```python
from build123d import *

# Parameters (mm, degrees)
BACK_PLATE_SKETCH_W    = 110
BACK_PLATE_SKETCH_H    = 66
BACK_PLATE_DEPTH       = 10
TOP_BOSS_44_DEPTH      = 20
TOP_BOSS_44_DEPTH_BACK = 20
TOP_BOSS_SKETCH_R      = 22
TOP_BOSS_SKETCH_R_2    = 11
PLATE_CUT_SKETCH_R     = 7.5
PLATE_CUT_DEPTH        = 20
BASE_BLOCK_DEPTH       = 64
BEARING_SADDLE_DEPTH   = 22
EAR_HOLES_SKETCH_R     = 6
EAR_HOLES_12_DEPTH     = 22
RIB_DEPTH              = 10
SIDE_PLATE_DEPTH       = 5
PAD_1_SKETCH_W         = 9.88210357
PAD_1_SKETCH_H         = 10
PAD_1_DEPTH            = 2
PAD_2_SKETCH_W         = 64
PAD_2_SKETCH_H         = 10
PAD_2_DEPTH            = 2


with BuildPart() as part:
    # Back Plate Sketch → Back Plate (new, symmetric)
    with BuildSketch(Plane(origin=(0, 0, 0), x_dir=(0, 0, -1), z_dir=(1, 0, 0))):
        Rectangle(BACK_PLATE_SKETCH_W, BACK_PLATE_SKETCH_H)
    extrude(amount=BACK_PLATE_DEPTH, both=True)

    # Plate Cut Sketch → Plate Cut (cut)
    with BuildSketch(Plane(origin=(10, 0, 0), x_dir=(0, 0, -1), z_dir=(1, 0, 0))):
        with Locations((42.5, 11)):
            Circle(PLATE_CUT_SKETCH_R)
        with Locations(Location((-42.5, 11, 0), (0, 0, 180))):
            Circle(PLATE_CUT_SKETCH_R)
    extrude(amount=-PLATE_CUT_DEPTH, mode=Mode.SUBTRACT)

    # Base Block Sketch → Base Block (add)
    with BuildSketch(Plane(origin=(10, 0, 0), x_dir=(0, 0, -1), z_dir=(1, 0, 0))):
        with BuildLine():
            Line((-32, -33), (-18, -33))
            ThreePointArc((-18, -33), (0, -15), (18, -33))
            Line((18, -33), (32, -33))
            ThreePointArc((32, -33), (0, -1), (-32, -33))
        make_face()
    extrude(amount=BASE_BLOCK_DEPTH)

    # Bearing Saddle Sketch → Bearing Saddle (add)
    with BuildSketch(Plane.XZ.offset(33)):
        with BuildLine():
            Line((27, 38), (27, 18))
            Line((27, 18), (57, 18))
            Line((57, 18), (57, 38))
            ThreePointArc((57, 38), (42, 53), (27, 38))
        make_face()
        with BuildLine():
            Line((27, -38), (27, -18))
            Line((27, -18), (57, -18))
            Line((57, -18), (57, -38))
            ThreePointArc((57, -38), (42, -53), (27, -38))
        make_face()
    extrude(amount=-BEARING_SADDLE_DEPTH)

    # Ear Holes Sketch → Ear Holes Ø12 (cut)
    with BuildSketch(Plane(origin=(0, -11, 0), x_dir=(1, 0, 0), z_dir=(0, 1, 0))):
        with Locations(Location((42, 38, 0), (0, 0, 270))):
            Circle(EAR_HOLES_SKETCH_R)
        with Locations(Location((42, -38, 0), (0, 0, 270))):
            Circle(EAR_HOLES_SKETCH_R)
    extrude(amount=-EAR_HOLES_12_DEPTH, mode=Mode.SUBTRACT)



with BuildPart() as body_2:
    # Top Boss Sketch → Top Boss Ø44 (new, two sides: drawn at the far end of the back side and taken through both)
    with BuildSketch(Plane(origin=(0, 0, 0), x_dir=(0, 0, -1), z_dir=(1, 0, 0)).offset(-TOP_BOSS_44_DEPTH_BACK)):
        with Locations((0, 67)):
            Circle(TOP_BOSS_SKETCH_R)
        with Locations((0, 67)):
            Circle(TOP_BOSS_SKETCH_R_2, mode=Mode.SUBTRACT)
    extrude(amount=TOP_BOSS_44_DEPTH + TOP_BOSS_44_DEPTH_BACK)


with BuildPart() as part_1:
    add(part.part)

    add(body_2.part)  # Rib merges body 2
    # Rib Sketch → Rib (add)
    with BuildSketch(Plane(origin=(10, 0, 0), x_dir=(0, 0, -1), z_dir=(1, 0, 0))):
        with BuildLine():
            Line((-22, 67), (-55, 33))
            Line((-55, 33), (55, 33))
            Line((55, 33), (22, 67))
            ThreePointArc((22, 67), (0, 45), (-22, 67))
        make_face()
    extrude(amount=-RIB_DEPTH)

    # Side Plate Sketch → Side Plate (add, symmetric)
    with BuildSketch(Plane.XY):
        Polygon((10, 44), (19.88210357, 44), (74, 0), (10, 0), align=None)
    extrude(amount=SIDE_PLATE_DEPTH, both=True)

    # Pad 1 Sketch → Pad 1 (add)
    with BuildSketch(Plane(origin=(0, 44, 0), x_dir=(1, 0, 0), z_dir=(0, 1, 0))):
        with Locations((14.941051785, 0)):
            Rectangle(PAD_1_SKETCH_W, PAD_1_SKETCH_H)
    extrude(amount=PAD_1_DEPTH)

    # Pad 2 Sketch → Pad 2 (add)
    with BuildSketch(Plane.XZ):
        with Locations((42, 0)):
            Rectangle(PAD_2_SKETCH_W, PAD_2_SKETCH_H)
    extrude(amount=PAD_2_DEPTH)


solid = part_1.part
```
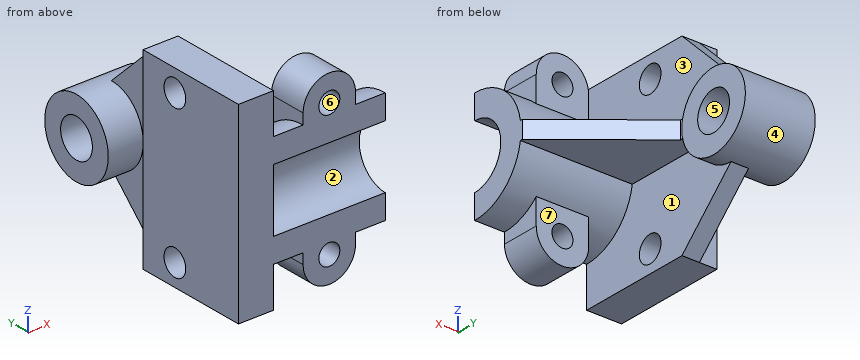
The model under review builds one solid part; all positions refer to its coordinate system, in mm. Face numbers are marked on the shaded views. A direction names the side the tool comes from. Give positions to 0.01 mm unless a question says otherwise; leave off trailing zeros. Loops run counter-clockwise (first coordinate to the right, second up) from the corner with the lowest first, then second, coordinate; pieces in that order, holes last. Notation, with made-up numbers: (81, -7.75) - (117, -7.75) arc R19 ccw to (117, 10.25) - close; hole circle Ø4 at (86, 21). An arc over 180 degrees is marked (long way). Answer as a JSON object with one key per item and string values.
Q1. To check wall thickness, follow line 1 along Y through (x, z) = (-6, 0); line 2 along Z through (x, y) = (3, 12.5); line 3 along Y through (x, z) = (15, -6). State the ranges of each line that lie inside material, in increasing order.
Worked out:
{"line 1": "y = -33 to 33, 45 to 56, 78 to 89", "line 2": "z = -55 to -49.85, -35.15 to 35.15, 49.85 to 55", "line 3": "y = -16.03 to -1.57, 45.83 to 57.78, 76.22 to 88.17"}
Q2. Insertion check: pin 1 (15 mm diameter, centred on x = 46.5, z = -43, fed in from +Y); pin 2 (15 mm diameter, centred on y = 12.5, z = 39, fed in from +X); pin 3 (5 mm diameter, centred on y = 9, z = 5, fed in from -X). Each pin has a flat end and moves straight along its axis. Give the tip position at first contact, or say it passes through.
Worked out:
{"pin 1": "stops at y = -11", "pin 2": "stops at x = 10", "pin 3": "stops at x = -10"}
Q3. Add section D-D on y = 62.5. State the section outline as (x, z) points, plus the area to 3 significant figures.
Worked out:
{"outline": "(-20, -21.53) - (0, -21.53) - (0, -26.37) - (10, -26.37) - (10, -21.53) - (20, -21.53) - (20, -10.04) - (-20, -10.04) - close; (-20, 10.04) - (20, 10.04) - (20, 21.53) - (10, 21.53) - (10, 26.37) - (0, 26.37) - (0, 21.53) - (-20, 21.53) - close", "area": "1,020 mm^2"}
Q4. For the marked faces 1, 2 and 3, list the 3-axis set-ups (+Z, -Z, +X, -X, +Y, -Y) from which the entire face can be reached by the end or side of a thin tool; tool diameter is ignored.
Worked out:
{"face 1": "-Z", "face 2": "+X, -Y", "face 3": "+Z"}
Q5. Mouldability with a two-part tool opening along Y and no side actions: class the marked faces 4, 5, 6 and 7 as +Y half, -Y half, draft (parallel to the pull), parting line (faces both ways), or undercut.
Worked out:
{"face 4": "undercut", "face 5": "undercut", "face 6": "draft", "face 7": "+Y half"}
Q6. Add section A-A on z = 0. State the section outline as (x, y) points, plus the area to 3 significant figures.
Worked out:
{"outline": "(-20, 45) - (0, 45) - (0, 33) - (-10, 33) - (-10, -33) - (10, -33) - (10, -15) - (74, -15) - (74, 0) - (19.88, 44) - (19.88, 45) - (20, 45) - (20, 56) - (-20, 56) - close; (-20, 78) - (20, 78) - (20, 89) - (-20, 89) - close", "area": "4,920 mm^2"}
Q7. Add section C-C on z = -42. State the section outline as (x, y) points.
Worked out:
{"outline": "(-10, -33) - (10, -33) - (10, 3.52) - (-10, 3.52) - close; (-10, 18.48) - (10, 18.48) - (10, 46.39) - (0, 46.39) - (0, 33) - (-10, 33) - close; (27.54, -33) - (37.53, -33) - (37.53, -11) - (27.54, -11) - close; (46.47, -33) - (56.46, -33) - (56.46, -11) - (46.47, -11) - close"}
Q8. Add section B-B on x = 7.5. State the section outline as (y, z) points.
Worked out:
{"outline": "(-33, -55) - (33, -55) - (67, -22) arc R22 ccw to (67, 22) - (33, 55) - (-33, 55) - close; hole circle Ø15 at (11, -42.5); hole circle Ø15 at (11, 42.5); hole circle Ø22 at (67, 0)"}
